Geometry: final body of the model. Coordinates: model frame, mm. Give positions to 0.01 mm unless a question says otherwise; leave off trailing zeros. Loops run counter-clockwise (first coordinate to the right, second up) from the corner with the lowest first, then second, coordinate; pieces in that order, holes last. Notation, with made-up numbers: (-28.75, 49) -> (-14.75, 49) arc R15 cw to (-14.75, 57) -> close; hole circle Ø9 at (49.5, -39). An arc over 180 degrees is marked (long way). Answer in a Markdown table with one row per item. Add a question column.
1) Section query A-A (y = 39). Return the cut outline in (x, z).
2) First-contact query: P1, Ø1.5, axis at x = -48, z = 36.5, coming from the -Y side; P2, Ø12, axis at x = -37.5, y = 0.5, coming from the -Z side; P3, Ø12, axis at x = -2.5, y = 26, coming from the +Z side. Flat tips, straight axial feed; report the tip coordinate or a pass-through.
3) Line query: line 1 (Y direction, x = 25, z = -28.5); line 2 (X direction, y = -30, z = 18.5); line 3 (Y direction, x = -3, z = -14). Output: solid intervals per line, ascending. Write a range as from..to.
```python
from build123d import *


with BuildPart() as part:
    # Top Half Profile → Spinning Top Revolve (revolve)
    with BuildSketch(Plane.XY, mode=Mode.PRIVATE) as spinning_top_revolve_sk:
        with BuildLine():
            ThreePointArc((66.699946845, -5), (69.123205901, -7.563423043), (66.570796819, -9.998280333))
            ThreePointArc((66.570796819, -9.998280333), (61.41938821, -9.943848556), (56.267998059, -10))
            ThreePointArc((56.267998059, -10), (41.561999586, -13.579345382), (30.145866595, -23.516649444))
            ThreePointArc((30.145866595, -23.516649444), (16.997479936, -43.6647974), (5.4, -64.743848539))
            ThreePointArc((5.4, -64.743848539), (3.55671587, -66.755540077), (0.931762793, -67.5))
            Line((0.931762793, -67.5), (0, -67.5))
            Line((0, -67.5), (0, 67.5))
            Line((0, 67.5), (1.02149392, 67.5))
            ThreePointArc((1.02149392, 67.5), (4.389313376, 66.19564502), (6, 62.963116845))
            Line((6, 62.963116845), (8.867384456, 31.532882589))
            ThreePointArc((8.867384456, 31.532882589), (9.414586997, 25.746129421), (10, 19.963116845))
            ThreePointArc((10, 19.963116845), (19.400534743, 6.856436897), (34, 0))
            ThreePointArc((34, 0), (50.309263809, -2.766240437), (66.699946845, -5))
        make_face()
    revolve(spinning_top_revolve_sk.sketch.rotate(Axis((0, 67.5, 0), (0, -1, 0)), 90), axis=Axis((0, 67.5, 0), (0, -1, 0)))


solid = part.part
```
Evaluation:
| question | item | result |
|---|---|---|
| 1 | outline | circle Ø16.37 at (0, 0) |
| 2 | P1 | y = -9.95 |
| 2 | P2 | z = -57.49 |
| 2 | P3 | z = 9.95 |
| 3 | line 1 | -15.79..-0.71 |
| 3 | line 2 | -17.81..17.81 |
| 3 | line 3 | -48.21..12.19 |
